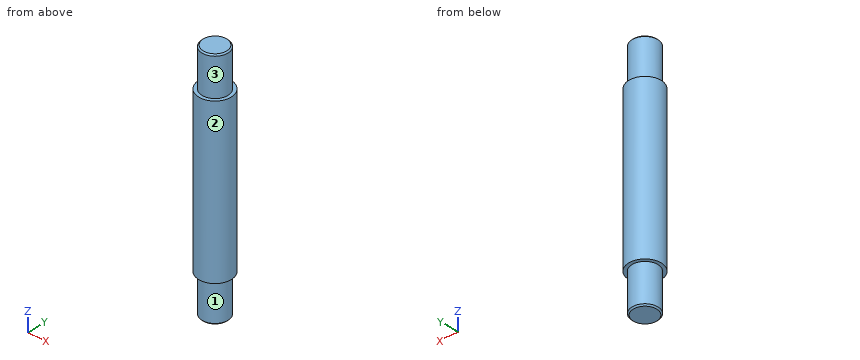
```python
from build123d import *

# Parameters (mm, degrees)
SKETCH1_R           = 12.5
BOSS_EXTRUDE1_DEPTH = 62.5
SKETCH2_R           = 10
BOSS_EXTRUDE2_DEPTH = 30
BOSS_EXTRUDE3_START = 30
SKETCH3_R           = 10
BOSS_EXTRUDE3_DEPTH = 30
CHAMFER1_SIZE       = 1


with BuildPart() as part:
    # Sketch1 → Boss-Extrude1 (new, symmetric)
    with BuildSketch(Plane.XY):
        Circle(SKETCH1_R)
    extrude(amount=BOSS_EXTRUDE1_DEPTH, both=True)

    # Sketch2 → Boss-Extrude2 (add)
    with BuildSketch(Plane.XY.offset(62.5)):
        Circle(SKETCH2_R)
    extrude(amount=BOSS_EXTRUDE2_DEPTH)

    # Sketch3 → Boss-Extrude3 (add)
    with BuildSketch(Plane(origin=(0, 0, -62.5), x_dir=(-1, 0, 0), z_dir=(0, 0, -1)).offset(BOSS_EXTRUDE3_START)):
        with Locations(Location((0, 0, 0), (0, 0, 180))):
            Circle(SKETCH3_R)
    extrude(amount=-BOSS_EXTRUDE3_DEPTH)

    # Chamfer1
    chamfer1_edges = [part.edges().sort_by_distance(p)[0] for p in [
        (-10, 0, -92.5),
        (-10, 0, 92.5),
    ]]
    chamfer(chamfer1_edges, length=CHAMFER1_SIZE)


solid = part.part
```
Geometry: final body of the model. Coordinates: model frame, mm. Face numbers are marked on the shaded views. A direction names the side the tool comes from. Coordinates: 2 decimals unless noted, no trailing zeros. Loops run counter-clockwise (first coordinate to the right, second up) from the corner with the lowest first, then second, coordinate; pieces in that order, holes last. Notation, with made-up numbers: (41.25, -29.5) -> (76.25, -29.5) arc R18 cw to (76.25, -24.5) -> close; hole circle Ø8 at (-13, 12). An arc over 180 degrees is marked (long way). Use a Markdown table: item, result. Add a question column.
(1) Section query C-C, the plane z = 76. Return loops of the section in (x, y), plus the area to 3 significant figures.
(2) Line query: line 1 along Y through (x, z) = (-0.5, 57.5); line 2 along Z through (x, y) = (7.5, 8); line 3 along Y through (x, z) = (7.5, 23). Output: solid intervals per line, ascending.
(3) Pin query (flat end, axial travel): pin 1 Ø10 at (x, z) = (1, -10.5) entering from +Y; pin 2 Ø10 at (x, z) = (0, -68.5) entering from -Y; pin 3 Ø1 at (x, y) = (9.5, -1) entering from -Z; pin 4 Ø1 at (y, z) = (7.5, -16.5) entering from -X. Return the tip coordinate at first contact, or that it passes through.
(4) Section query D-D, the plane z = -35. Return loops of the section in (x, y), plus the area to 3 significant figures.
(5) Section query A-A, the plane x = 0. Return loops of the section in (y, z), plus the area to 3 significant figures.
(6) Access query for the marked faces 1, 2 and 3. Directions: +Z, -Z, +X, -X, +Y, -Y. A direction counts if a zero-diameter tool reaches every point of the face in a straight line with its end or side. Return the directions, or none.
Answer:
| question | item | result |
|---|---|---|
| 1 | outline | circle Ø20 at (0, 0) |
| 1 | area | 314 mm^2 |
| 2 | line 1 | y = -12.49 to 12.49 |
| 2 | line 2 | z = -62.5 to 62.5 |
| 2 | line 3 | y = -10 to 10 |
| 3 | pin 1 | stops at y = 12.5 |
| 3 | pin 2 | stops at y = -10 |
| 3 | pin 3 | stops at z = -92.45 |
| 3 | pin 4 | stops at x = -10.36 |
| 4 | outline | circle Ø25 at (0, 0) |
| 4 | area | 491 mm^2 |
| 5 | outline | (-12.5, -62.5) -> (-10, -62.5) -> (-10, -91.5) -> (-9, -92.5) -> (9, -92.5) -> (10, -91.5) -> (10, -62.5) -> (12.5, -62.5) -> (12.5, 62.5) -> (10, 62.5) -> (10, 91.5) -> (9, 92.5) -> (-9, 92.5) -> (-10, 91.5) -> (-10, 62.5) -> (-12.5, 62.5) -> close |
| 5 | area | 4,320 mm^2 |
| 6 | face 1 | -Z |
| 6 | face 2 | +Z, -Z |
| 6 | face 3 | +Z |
